For this review, take the finished solid that the model builds, in its own axes (mm). Face numbers are marked on the shaded views. A direction names the side the tool comes from. Coordinates: 2 decimals unless noted, no trailing zeros. Write each loop counter-clockwise with the first axis right and the second up, starting at its lowest first coordinate (ties: lowest second). Pieces come first, ordered by that corner, then holes. Notation, with made-up numbers: M 6.5,27 L 65.5,27 A28 ccw 65.5,54 Z; hole C 2,37 d2. An arc over 180 degrees is marked long. Return JSON: item names as keys, results as strings.
```python
from build123d import *

# Parameters (mm, degrees)
SKETCH_1_W                = 130
SKETCH_1_H                = 14
EXTRUDE_1_DEPTH           = 12.5
SKETCH_2_W                = 11.5
SKETCH_2_H                = 1.5
CUT_EXTRUDE_1_DEPTH       = 131.787040642
CHAMFER_3_SIZE            = 2
CHAMFER_3_SIZE2           = 5
CHAMFER_4_SIZE            = 5
CHAMFER_4_SIZE2           = 2
HOLE_WIZARD_1_D           = 3.4
HOLE_WIZARD_1_CBORE_D     = 6
HOLE_WIZARD_1_CBORE_DEPTH = 3.4


with BuildPart() as part:
    # 草图1 → 凸台-拉伸1 (new body)
    with BuildSketch(Plane.XY):
        Rectangle(SKETCH_1_W, SKETCH_1_H)
    extrude(amount=EXTRUDE_1_DEPTH)

    # 草图2 → 切除-拉伸1 (cut, through all)
    with BuildSketch(Plane(origin=(65, 0, 0), x_dir=(0, 0, -1), z_dir=(1, 0, 0))):
        with Locations((-6.75, 6.25)):
            Rectangle(SKETCH_2_W, SKETCH_2_H)
    extrude(amount=-CUT_EXTRUDE_1_DEPTH, mode=Mode.SUBTRACT)

    # 倒角3
    chamfer_3_edges = [part.edges().sort_by_distance(p)[0] for p in [
        (65, 5.5, 6.75),
    ]]
    chamfer_3_side = [part.faces().sort_by_distance(p)[0] for p in [
        (65, -0.683438986, 6.195324881),
    ]]
    chamfer(chamfer_3_edges, length=CHAMFER_3_SIZE, length2=CHAMFER_3_SIZE2, reference=chamfer_3_side[0])

    # 倒角4
    chamfer_4_edges = [part.edges().sort_by_distance(p)[0] for p in [
        (-65, 5.5, 6.75),
    ]]
    chamfer_4_side = [part.faces().sort_by_distance(p)[0] for p in [
        (-2.5, 5.5, 6.75),
    ]]
    chamfer(chamfer_4_edges, length=CHAMFER_4_SIZE, length2=CHAMFER_4_SIZE2, reference=chamfer_4_side[0])

    # 打孔尺寸根据内六角圆柱头螺钉的类型1 (through all)
    with Locations(Plane(origin=(0, 0, 0), x_dir=(-1, 0, 0), z_dir=(0, 0, -1))):
        with Locations((-40, 0), (40, 0)):
            CounterBoreHole(HOLE_WIZARD_1_D / 2, HOLE_WIZARD_1_CBORE_D / 2, HOLE_WIZARD_1_CBORE_DEPTH)


solid = part.part
```
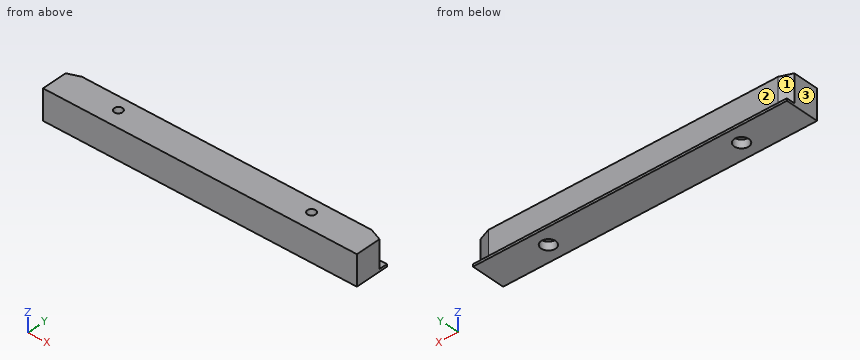
1. Wall thickness on L1, parallel to X at y = -1, z = 1; L2, parallel to Y at x = 40, z = 6.25; L3, parallel to Y at x = 40, z = 0.9: over which ranges is each line inside the solid? List them lowest first. Write a range as from..to.
Checks:
{"L1": "-65..-42.83, -37.17..37.17, 42.83..65", "L2": "-7..-1.7, 1.7..5.5", "L3": "-7..-3, 3..7"}
2. We need section B-B (y = 0). State the section outline as (x, z) points, plus the area to 3 significant figures.
Checks:
{"outline": "M -65,0 L -43,0 L -43,3.4 L -41.7,3.4 L -41.7,12.5 L -65,12.5 Z; M -38.3,3.4 L -37,3.4 L -37,0 L 37,0 L 37,3.4 L 38.3,3.4 L 38.3,12.5 L -38.3,12.5 Z; M 41.7,3.4 L 43,3.4 L 43,0 L 65,0 L 65,12.5 L 41.7,12.5 Z", "area": "1,520 mm2"}
3. Clearance check with flat-ended pins moving along their axes: pin 1 Ø2 at (x, y) = (40, 0) entering from +Z; pin 2 Ø5.5 at (x, y) = (40, 0) entering from -Z; pin 3 Ø1 at (x, z) = (38, 10.5) entering from +Y. State where each tip first meets the part, or that it passes through.
Checks:
{"pin 1": "through", "pin 2": "z = 3.4", "pin 3": "y = 5.5"}
4. We need section A-A (x = 40). State the section outline as (y, z) points, plus the area to 3 significant figures.
Checks:
{"outline": "M -7,0 L -3,0 L -3,3.4 L -1.7,3.4 L -1.7,12.5 L -7,12.5 Z; M 1.7,3.4 L 3,3.4 L 3,0 L 7,0 L 7,1 L 5.5,1 L 5.5,12.5 L 1.7,12.5 Z", "area": "106 mm2"}
5. We need section C-C (z = 8.5). State the section outline as (x, y) points, plus the area to 3 significant figures.
Checks:
{"outline": "M -65,-7 L 65,-7 L 65,3.5 L 60,5.5 L -60,5.5 L -65,3.5 Z; hole C -40,0 d3.4; hole C 40,0 d3.4", "area": "1,600 mm2"}
6. We need section D-D (x = -10). State the section outline as (y, z) points, plus the area to 3 significant figures.
Checks:
{"outline": "M -7,0 L 7,0 L 7,1 L 5.5,1 L 5.5,12.5 L -7,12.5 Z", "area": "158 mm2"}
7. For the marked faces 1, 2 and 3, list the 3-axis set-ups (+Z, -Z, +X, -X, +Y, -Y) from which the entire face can be reached by the end or side of a thin tool; tool diameter is ignored.
Checks:
{"face 1": "+Z, -X, +Y", "face 2": "+Z, +X, -X, +Y", "face 3": "+Z, -Z, -X, +Y, -Y"}
